Input: part model. Units: mm. Frame: model coordinates. A direction names the side the tool comes from. Round coordinates to 2 decimals unless told otherwise and drop trailing zeros. Write each loop counter-clockwise with the first axis right and the second up, starting at its lowest first coordinate (ties: lowest second). Pieces come first, ordered by that corner, then holes. Notation, with made-up numbers: (-8, -31) - (46, -31) arc R10 cw to (46, -17) - close; hole circle Ø5 at (-11, 77). An arc over 180 degrees is marked (long way). One line per item, written item: value. Start each with the question number.
```python
from build123d import *

# Parameters (mm, degrees)
SKETCH1_R           = 1.6
BOSS_EXTRUDE1_DEPTH = 5
SKETCH2_R           = 2.9
CUT_EXTRUDE1_DEPTH  = 3.2


with BuildPart() as part:
    # Sketch1 → Boss-Extrude1 (new body)
    with BuildSketch(Plane(origin=(0, 0, 0), x_dir=(1, 0, 0), z_dir=(0, 1, 0))):
        with BuildLine():
            Line((-40, -35), (40, -35))
            ThreePointArc((40, -35), (43.535533906, -33.535533906), (45, -30))
            Line((45, -30), (45, 30))
            ThreePointArc((45, 30), (43.535533906, 33.535533906), (40, 35))
            Line((40, 35), (-40, 35))
            ThreePointArc((-40, 35), (-43.535533906, 33.535533906), (-45, 30))
            Line((-45, 30), (-45, -30))
            ThreePointArc((-45, -30), (-43.535533906, -33.535533906), (-40, -35))
        make_face()
        with Locations(Location((-41, 31, 0), (0, 0, 270))):
            Circle(SKETCH1_R, mode=Mode.SUBTRACT)
        with Locations(Location((-41, -31, 0), (0, 0, 270))):
            Circle(SKETCH1_R, mode=Mode.SUBTRACT)
        with Locations(Location((41, -31, 0), (0, 0, 270))):
            Circle(SKETCH1_R, mode=Mode.SUBTRACT)
        with Locations(Location((41, 31, 0), (0, 0, 270))):
            Circle(SKETCH1_R, mode=Mode.SUBTRACT)
    extrude(amount=BOSS_EXTRUDE1_DEPTH)

    # Sketch2 → Cut-Extrude1 (cut)
    with BuildSketch(Plane(origin=(0, 5, 0), x_dir=(1, 0, 0), z_dir=(0, 1, 0))):
        with Locations(Location((41, 31, 0), (0, 0, 270))):
            Circle(SKETCH2_R)
        with Locations(Location((-41, 31, 0), (0, 0, 270))):
            Circle(SKETCH2_R)
        with Locations(Location((-41, -31, 0), (0, 0, 270))):
            Circle(SKETCH2_R)
        with Locations(Location((41, -31, 0), (0, 0, 270))):
            Circle(SKETCH2_R)
    extrude(amount=-CUT_EXTRUDE1_DEPTH, mode=Mode.SUBTRACT)


solid = part.part
```
Q1. Pull-direction query (X, two-part tool) for faces 1 (the flat face through (39.75, 1.8, 32.25)), 2 (the cylindrical face through (-43, 2, -34)), 3 (the cylindrical face through (43, 2, 34)); classes: pulls with the +X half, pulls with the -X half, needs draft (parallel to the pull), parting line crosses it, or undercut.
Q2. Contact query for flat-ended pins moving along their axis: pin 1 Ø4.5 at (x, z) = (-41, 31) entering from +Y; pin 2 Ø2.5 at (x, z) = (41, -31) entering from +Y. Output: stop coordinate, or through.
Q3. Cut plane B-B, the plane x = 41. Output: boundary loops of the cut face in (y, z), and give its area (3 significant figures).
Q4. Access query for faces 4 (the flat face through (-42.25, 1.8, -29.75)), 5 (the cylindrical face through (40.03, 0.89, 29.73)). Directions: +Z, -Z, +X, -X, +Y, -Y. A direction counts if a zero-diameter tool reaches every point of the face in a straight line with its end or side. Return the directions, or none.
Q5. Material intervals for probe 1 along X at (y, z) = (2.2, 32); probe 2 along X at (y, z) = (3.75, -31); probe 3 along Z at (x, y) = (-41, 0.6), sorted ascending. Write a range as from..to.
Q6. Cut plane C-C, the plane z = -31. Output: boundary loops of the cut face in (x, y), and give its area (3 significant figures).
Q7. Cut plane A-A, the plane y = 2.75. Output: boundary loops of the cut face in (x, z).
A:
1. face 1: undercut
1. face 2: pulls with the -X half
1. face 3: pulls with the +X half
2. pin 1: stops at y = 1.8
2. pin 2: passes through
3. outline: (0, -34.9) - (5, -34.9) - (5, -33.9) - (1.8, -33.9) - (1.8, -32.6) - (0, -32.6) - close; (0, -29.4) - (1.8, -29.4) - (1.8, -28.1) - (5, -28.1) - (5, 28.1) - (1.8, 28.1) - (1.8, 29.4) - (0, 29.4) - close; (0, 32.6) - (1.8, 32.6) - (1.8, 33.9) - (5, 33.9) - (5, 34.9) - (0, 34.9) - close
3. area: 300 mm²
4. face 4: +Y
4. face 5: +Y, -Y
5. probe 1: x = -44.58..-43.72, -38.28..38.28, 43.72..44.58
5. probe 2: x = -44.9..-43.9, -38.1..38.1, 43.9..44.9
5. probe 3: z = -34.9..-32.6, -29.4..29.4, 32.6..34.9
6. outline: (-44.9, 0) - (-42.6, 0) - (-42.6, 1.8) - (-43.9, 1.8) - (-43.9, 5) - (-44.9, 5) - close; (-39.4, 0) - (39.4, 0) - (39.4, 1.8) - (38.1, 1.8) - (38.1, 5) - (-38.1, 5) - (-38.1, 1.8) - (-39.4, 1.8) - close; (42.6, 0) - (44.9, 0) - (44.9, 5) - (43.9, 5) - (43.9, 1.8) - (42.6, 1.8) - close
6. area: 400 mm²
7. outline: (-45, -30) arc R5 ccw to (-40, -35) - (40, -35) arc R5 ccw to (45, -30) - (45, 30) arc R5 ccw to (40, 35) - (-40, 35) arc R5 ccw to (-45, 30) - close; hole circle Ø5.8 at (-41, -31); hole circle Ø5.8 at (-41, 31); hole circle Ø5.8 at (41, -31); hole circle Ø5.8 at (41, 31)
